```python
from build123d import *


with BuildPart() as part:
    # Sketch1 → Revolve1 (revolve)
    with BuildSketch(Plane.XY, mode=Mode.PRIVATE) as revolve1_sk:
        with BuildLine():
            Line((3, 0), (21.5, 0))
            Line((21.5, 0), (14.481102974, 4.822150816))
            ThreePointArc((14.481102974, 4.822150816), (14.13417871, 5.491793096), (14.498167484, 6.152315163))
            Line((14.498167484, 6.152315163), (21.957245997, 11))
            Line((21.957245997, 11), (23, 11))
            ThreePointArc((23, 11), (24, 12), (23, 13))
            Line((23, 13), (22.361328191, 13))
            Line((22.361328191, 13), (8.75, 25))
            Line((8.75, 25), (8.75, 29.2))
            Line((8.75, 29.2), (8, 29.2))
            Line((8, 29.2), (9, 29.777350269))
            Line((9, 29.777350269), (9, 32.622649731))
            Line((9, 32.622649731), (8, 33.2))
            Line((8, 33.2), (7, 33.2))
            Line((7, 33.2), (7, 34))
            Line((7, 34), (3, 34))
            Line((3, 34), (3, 0))
        make_face()
    revolve(revolve1_sk.sketch.rotate(Axis((0, 0, 0), (0, 1, 0)), 270), axis=Axis((0, 0, 0), (0, 1, 0)))


solid = part.part
```
The model under review builds one solid part; all positions refer to its coordinate system, in mm. A direction names the side the tool comes from. Give positions to 0.01 mm unless a question says otherwise; leave off trailing zeros. Loops run counter-clockwise (first coordinate to the right, second up) from the corner with the lowest first, then second, coordinate; pieces in that order, holes last. Notation, with made-up numbers: (39, 58.5) - (53, 58.5) arc R19 cw to (53, 92.5) - close; hole circle Ø4 at (-2.75, 51). An arc over 180 degrees is marked (long way). Answer as a JSON object with one key per item and string values.
Q1. Insertion check: pin 1 (5 mm diameter, centred on y = 7.5, z = 4, fed in from +X); pin 2 (3 mm diameter, centred on y = 6.5, z = 7.5, fed in from -X); pin 3 (12 mm diameter, centred on x = -3.5, y = 23, fed in from +Z). Each pin has a flat end and moves straight along its axis. Give the tip position at first contact, or say it passes through.
Worked out:
{"pin 1": "stops at x = 20.05", "pin 2": "stops at x = -15.73", "pin 3": "stops at z = 17.56"}
Q2. Add section C-C on y = 16.5. State the section outline as (x, z) points, plus the area to 3 significant figures.
Worked out:
{"outline": "circle Ø36.78 at (0, 0); hole circle Ø6 at (0, 0)", "area": "1,030 mm^2"}
Q3. To check wall thickness, follow line 1 along X through (y, z) = (26, 0); line 2 along Y through (x, z) = (13, 8); line 3 along X through (y, z) = (22, 0). State the ranges of each line that lie inside material, in increasing order.
Worked out:
{"line 1": "x = -8.75 to -3, 3 to 8.75", "line 2": "y = 0 to 4.28, 6.65 to 19.26", "line 3": "x = -12.15 to -3, 3 to 12.15"}
Q4. For faces 1 (the flat face through (-19, 11, -12)), 2 (the flat face through (-6, 33.2, 4)), 3 (the cylindrical face through (-5.324, 27.129, -6.944)), list the 3-axis set-ups (+Z, -Z, +X, -X, +Y, -Y) from which the entire face can be reached by the end or side of a thin tool; tool diameter is ignored.
Worked out:
{"face 1": "-Y", "face 2": "+Y", "face 3": "none"}
Q5. Add section D-D on y = 8. State the section outline as (x, z) points.
Worked out:
{"outline": "circle Ø34.68 at (0, 0); hole circle Ø6 at (0, 0)"}
Q6. Mouldability with a two-part tool opening along X and no side actions: class faces 4 (the conical face through (-5.726, 24.417, -7.468)), 5 (the flat face through (22.3, 13, -3.5)), 6 (the cylindrical face through (0.9, 16.76, 2.86)) as +X half, -X half, draft (parallel to the pull), parting line (faces both ways), or undercut.
Worked out:
{"face 4": "parting line", "face 5": "draft", "face 6": "undercut"}
